```python
from build123d import *

# Parameters (mm, degrees)
EXTRUDE_1_DEPTH     = 15
SKETCH_4_R          = 39.55
SKETCH_4_R_2        = 18
CUT_EXTRUDE_1_DEPTH = 1.875
CUT_EXTRUDE_1_DRAFT = -60
CHAMFER_1_SIZE      = 1.333333333


with BuildPart() as part:
    # 草图3 → 凸台-拉伸1 (new body)
    with BuildSketch(Plane(origin=(0, 0, 0), x_dir=(0, 0, -1), z_dir=(1, 0, 0))):
        Polygon((18, 10.392304845), (0, 20.784609691), (-18, 10.392304845), (-18, -10.392304845), (0, -20.784609691), (18, -10.392304845), align=None)
    extrude(amount=EXTRUDE_1_DEPTH)


with BuildPart() as cut_extrude_1_tool:
    # 草图4 → 切除-拉伸1 (with draft: the straight prism first)
    with BuildSketch(Plane.ZY):
        Circle(SKETCH_4_R)
        Circle(SKETCH_4_R_2, mode=Mode.SUBTRACT)
    extrude(amount=-CUT_EXTRUDE_1_DEPTH)
    # 切除-拉伸1: the draft: its side faces are tilted about the plane it starts from
    cut_extrude_1_sides = [cut_extrude_1_tool.faces().sort_by_distance(p)[0] for p in [
        (0.9375, 0, -39.55),
        (0.9375, 0, -18),
    ]]
    draft(cut_extrude_1_sides, Plane.ZY, CUT_EXTRUDE_1_DRAFT)


with BuildPart() as part_1:
    add(part.part)

    # 切除-拉伸1: cut by cut_extrude_1_tool
    add(cut_extrude_1_tool.part, mode=Mode.SUBTRACT)

    # 草图6 → 旋转2 (revolve)
    with BuildSketch(Plane.XY, mode=Mode.PRIVATE) as revolve_2_sk:
        with BuildLine():
            Line((24, 12), (75, 12))
            Line((75, 12), (75, 0))
            Line((75, 0), (15, 0))
            Line((15, 0), (15, 13.22575))
            ThreePointArc((15, 13.22575), (15.76171636, 11.561015736), (17.519400155, 11.049059039))
            Line((17.519400155, 11.049059039), (24, 12))
        make_face()
    revolve(revolve_2_sk.sketch.rotate(Axis((15, 0, 0), (1, 0, 0)), 180), axis=Axis((15, 0, 0), (1, 0, 0)))

    # 倒角1
    chamfer_1_edges = [part_1.edges().sort_by_distance(p)[0] for p in [
        (75, 12, 0),
    ]]
    chamfer(chamfer_1_edges, length=CHAMFER_1_SIZE)

    # 草图8 → 切除-旋转2 (revolve, cut)
    with BuildSketch(Plane.XY, mode=Mode.PRIVATE) as cut_revolve_2_sk:
        Polygon((15, 16.525), (14.2, 17.325), (14.2, 39.55), (15, 39.55), align=None)
    revolve(cut_revolve_2_sk.sketch.rotate(Axis((0, 0, 0), (1, 0, 0)), 180), axis=Axis((0, 0, 0), (1, 0, 0)), mode=Mode.SUBTRACT)


solid = part_1.part
```
Input: part model. Units: mm. Frame: model coordinates. A direction names the side the tool comes from. Coordinates: 2 decimals unless noted, no trailing zeros. Write each loop counter-clockwise with the first axis right and the second up, starting at its lowest first coordinate (ties: lowest second). Pieces come first, ordered by that corner, then holes.
1) Set-up query: faces 1 (the flat face through (7.001, -15.661, -8.874)), 2 (the flat face through (15, 14, 0)). Return all of +Z, -Z, +X, -X, +Y, -Y with unobstructed straight access to the full face (end or side cutting, diameter ignored); none if empty.
2) Material intervals for line 1 along X through (y, z) = (5.5, -15.5); line 2 along Z through (x, y) = (59, -5.5); line 3 along X through (y, z) = (-17.5, -3.5), sorted ascending.
3) Mould query, pull axis Y, two halves, no side actions, for faces 3 (the flat face through (7.001, -15.516, 9.126)), 4 (the cylindrical face through (49.181, -11.446, -3.604)), 5 (the flat face through (75, 0, 0)). Classes: pulls with the +Y half, pulls with the -Y half, needs draft (parallel to the pull), parting line crosses it, or undercut.
4) Section A-A on x = 5. Output: boundary loops of the cut face in (y, z), and give its area (3 significant figures).
5) Pin query (flat end, axial travel): pin 1 Ø5 at (x, z) = (28, -11) entering from -Y; pin 2 Ø6 at (x, z) = (28.5, 11) entering from -Y; pin 3 Ø2 at (x, y) = (53.5, -10) entering from +Z; pin 4 Ø5 at (y, z) = (-5.5, -10.5) entering from +X. Return the tip coordinate at first contact, or that it passes through.
6) Section B-B on x = 49.5. Output: boundary loops of the cut face in (y, z).
Check result:
1. face 1: -Z, +X, -X, -Y
1. face 2: +X
2. line 1: x = 0 to 15
2. line 2: z = -10.67 to 10.67
2. line 3: x = 0 to 14.2
3. face 3: pulls with the -Y half
3. face 4: parting line crosses it
3. face 5: needs draft
4. outline: (-20.78, 0) - (-10.39, -18) - (10.39, -18) - (20.78, 0) - (10.39, 18) - (-10.39, 18) - close
4. area: 1,120 mm2
5. pin 1: stops at y = -8.47
5. pin 2: stops at y = -8.94
5. pin 3: stops at z = 7.94
5. pin 4: stops at x = 75
6. outline: circle Ø24 at (0, 0)
